The model under review builds one solid part; all positions refer to its coordinate system, in mm. A direction names the side the tool comes from. Give positions to 0.01 mm unless a question says otherwise; leave off trailing zeros. Write each loop counter-clockwise with the first axis right and the second up, starting at its lowest first coordinate (ties: lowest second). Pieces come first, ordered by that corner, then holes. Notation, with made-up numbers: (-4.75, 29) -> (30.25, 29) arc R36 ccw to (30.25, 63) -> close; hole circle Ø8 at (37.25, 15.5). An arc over 180 degrees is marked (long way). Use CSV: the item, a comma, the result in double quotes.
```python
from build123d import *

# Parameters (mm, degrees)
BASE_PLATE_DEPTH       = 8
BASE_HOLE_SKETCH_R     = 8
BASE_HOLE_DEPTH        = 8
UPRIGHT_ARM_DEPTH      = 32
BOSS_MOUNT_DEPTH       = 10
CYLINDER_START         = 10
CYLINDER_BOSS_SKETCH_R = 15
CYLINDER_BOSS_DEPTH    = 10
BOSS_BORE_SKETCH_R     = 10
BOSS_BORE_DEPTH        = 20
GUSSET_DEPTH           = 40
GUSSET_TRIM_1_DEPTH    = 14
GUSSET_TRIM_2_DEPTH    = 14


with BuildPart() as part:
    # Base Plate Sketch → Base Plate (new body)
    with BuildSketch(Plane.XY):
        with BuildLine():
            Line((0, 18), (56, 18))
            ThreePointArc((56, 18), (74, 0), (56, -18))
            Line((56, -18), (0, -18))
            ThreePointArc((0, -18), (-18, 0), (0, 18))
        make_face()
    extrude(amount=BASE_PLATE_DEPTH)

    # Base Hole Sketch → Base Hole (cut)
    with BuildSketch(Plane.XY.offset(8)):
        Circle(BASE_HOLE_SKETCH_R)
        with Locations((56, 0)):
            Circle(BASE_HOLE_SKETCH_R)
    extrude(amount=-BASE_HOLE_DEPTH, mode=Mode.SUBTRACT)

    # Upright Arm Sketch → Upright Arm (add)
    with BuildSketch(Plane.XY.offset(8)):
        Polygon((28, 18), (8, 18), (8, 8), (48, 8), (48, 18), align=None)
    extrude(amount=UPRIGHT_ARM_DEPTH)

    # Boss Mount Sketch → Boss Mount (add)
    with BuildSketch(Plane.XY.offset(40)):
        with BuildLine():
            Line((13.388373349, 53.391219044), (13.041195377, 51.110929457))
            ThreePointArc((13.041195377, 51.110929457), (27.444153502, 35.010302382), (43, 50))
            ThreePointArc((43, 50), (42.989697618, 50.555846498), (42.958804623, 51.110929457))
            Line((42.958804623, 51.110929457), (42.611626651, 53.391219044))
            ThreePointArc((42.611626651, 53.391219044), (28, 65), (13.388373349, 53.391219044))
        make_face()
        with BuildLine():
            Line((13.041195377, 51.110929457), (8, 18))
            Line((8, 18), (48, 18))
            Line((48, 18), (42.958804623, 51.110929457))
            ThreePointArc((42.958804623, 51.110929457), (42.989697618, 50.555846498), (43, 50))
            ThreePointArc((43, 50), (27.444153502, 35.010302382), (13.041195377, 51.110929457))
        make_face()
    extrude(amount=-BOSS_MOUNT_DEPTH)

    # Cylinder Boss Sketch → Cylinder Boss (add)
    with BuildSketch(Plane.XY.offset(40).offset(CYLINDER_START)):
        with Locations((28, 50)):
            Circle(CYLINDER_BOSS_SKETCH_R)
    extrude(amount=-CYLINDER_BOSS_DEPTH)

    # Boss Bore Sketch → Boss Bore (cut)
    with BuildSketch(Plane.XY.offset(50)):
        with Locations((28, 50)):
            Circle(BOSS_BORE_SKETCH_R)
    extrude(amount=-BOSS_BORE_DEPTH, mode=Mode.SUBTRACT)

    # Gusset Sketch → Gusset (add)
    with BuildSketch(Plane(origin=(48, 0, 0), x_dir=(0, 0, -1), z_dir=(1, 0, 0))):
        Polygon((-40, 8), (-8, -18), (-8, 8), align=None)
    extrude(amount=-GUSSET_DEPTH)

    # Gusset Trim 1 Sketch → Gusset Trim 1 (cut)
    with BuildSketch(Plane(origin=(48, 0, 0), x_dir=(0, 0, -1), z_dir=(1, 0, 0))):
        Polygon((-40, 8), (-8, 8), (-8, -18), align=None)
    extrude(amount=-GUSSET_TRIM_1_DEPTH, mode=Mode.SUBTRACT)

    # Gusset Trim 2 Sketch → Gusset Trim 2 (cut)
    with BuildSketch(Plane.ZY.offset(-8)):
        Polygon((40, 8), (8, 8), (8, -18), align=None)
    extrude(amount=-GUSSET_TRIM_2_DEPTH, mode=Mode.SUBTRACT)


solid = part.part
```
Q1. To check wall thickness, follow probe 1 along X at (y, z) = (6, 3); probe 2 along Y at (x, z) = (56, 3); probe 3 along Y at (x, z) = (28, 44). State the ranges of each line that lie inside material, in increasing order.
Derived:
probe 1,"x = -16.97 to -5.29, 5.29 to 50.71, 61.29 to 72.97"
probe 2,"y = -18 to -8, 8 to 18"
probe 3,"y = 35 to 40, 60 to 65"
Q2. Consider section C-C (y = 0). Write out the cut boundary in (x, z).
Derived:
outline,"(-18, 0) -> (-8, 0) -> (-8, 8) -> (-18, 8) -> close; (8, 0) -> (48, 0) -> (48, 8) -> (34, 8) -> (34, 30.15) -> (22, 30.15) -> (22, 8) -> (8, 8) -> close; (64, 0) -> (74, 0) -> (74, 8) -> (64, 8) -> close"
Q3. Consider section A-A (x = 28). Write out the cut boundary in (y, z).
Derived:
outline,"(-18, 0) -> (18, 0) -> (18, 30) -> (40, 30) -> (40, 50) -> (35, 50) -> (35, 40) -> (8, 40) -> (-18, 8) -> close; (60, 30) -> (65, 30) -> (65, 50) -> (60, 50) -> close"
Q4. Consider section B-B (y = 50). Write out the cut boundary in (x, z), then the cut area to 3 significant figures.
Derived:
outline,"(12.87, 30) -> (18, 30) -> (18, 50) -> (13, 50) -> (13, 40) -> (12.87, 40) -> close; (38, 30) -> (43.13, 30) -> (43.13, 40) -> (43, 40) -> (43, 50) -> (38, 50) -> close"
area,"203 mm2"
Q5. Machinability: for faces 4 (the flat face through (48, 13, 24)), 5 (the flat face through (8, 13, 24)), 6 (the flat face through (28, 18, 15)), 7 (the flat face through (15, 8, 24)), which of the approach directions +Z, -Z, +X, -X, +Y, -Y give a long, thin tool a straight path to every point of the face, cutting with its end or side? Answer none if there is none.
Derived:
face 4,"+Z, +X, +Y, -Y"
face 5,"+Z, -X, +Y, -Y"
face 6,"-Z, +X, -X, +Y"
face 7,"+Z, -X, -Y"
Q6. The part is to be moulded in two halves that separate along X. For faces 1 (the cylindrical face through (74, 0, 4)), 2 (the cylindrical face through (32.614, 41.128, 40.14)), 3 (the flat face through (28, 37, 30)), say which applies: pulls with the +X half, pulls with the -X half, needs draft (parallel to the pull), parting line crosses it, or undercut.
Derived:
face 1,"pulls with the +X half"
face 2,"undercut"
face 3,"needs draft"
Q7. Insertion check: pin 1 (4 mm diameter, centred on x = 18.5, z = 22.5, fed in from -Y); pin 2 (11 mm diameter, centred on y = 11, z = 19.5, fed in from +X); pin 3 (4 mm diameter, centred on x = 23.5, z = 10, fed in from +Y). Each pin has a flat end and moves straight along its axis. Give the tip position at first contact, or say it passes through.
Derived:
pin 1,"stops at y = 8"
pin 2,"stops at x = 48"
pin 3,"stops at y = 18"
Q8. Consider section D-D (z = 20). Write out the cut boundary in (x, y).
Derived:
outline,"(8, 8) -> (22, 8) -> (22, -8.25) -> (34, -8.25) -> (34, 8) -> (48, 8) -> (48, 18) -> (8, 18) -> close"
